from build123d import *

# Parameters (mm, degrees)
SKETCH1_W           = 600
SKETCH1_H           = 300
BOSS_EXTRUDE1_DEPTH = 60
SKETCH2_R           = 42.5
SKETCH2_W           = 550
SKETCH2_H           = 60
CUT_EXTRUDE1_DEPTH  = 34
SKETCH3_W           = 580
SKETCH3_H           = 280
CUT_EXTRUDE2_DEPTH  = 4
SKETCH4_W           = 15
SKETCH4_H           = 96.703930486
CUT_EXTRUDE3_DEPTH  = 4
LPATTERN1_COUNT     = 3
LPATTERN1_PITCH     = 100
LPATTERN1_COL_COUNT = 3
LPATTERN1_COL_PITCH = 100


with BuildPart() as part:
    # Sketch1 → Boss-Extrude1 (new body)
    with BuildSketch(Plane(origin=(0, 0, 0), x_dir=(1, 0, 0), z_dir=(0, 1, 0))):
        Rectangle(SKETCH1_W, SKETCH1_H)
    extrude(amount=BOSS_EXTRUDE1_DEPTH)

    # Sketch2 → Cut-Extrude1 (cut)
    with BuildSketch(Plane(origin=(0, 60, 0), x_dir=(1, 0, 0), z_dir=(0, 1, 0))):
        with Locations(Location((0, 80, 0), (0, 0, 270))):
            Circle(SKETCH2_R)
        with Locations(Location((0, -80, 0), (0, 0, 90))):
            Circle(SKETCH2_R)
        with Locations(Location((-100, 80, 0), (0, 0, 270))):
            Circle(SKETCH2_R)
        with Locations(Location((-200, 80, 0), (0, 0, 270))):
            Circle(SKETCH2_R)
        with Locations(Location((200, 80, 0), (0, 0, 90))):
            Circle(SKETCH2_R)
        with Locations(Location((100, 80, 0), (0, 0, 90))):
            Circle(SKETCH2_R)
        with Locations(Location((200, -80, 0), (0, 0, 270))):
            Circle(SKETCH2_R)
        with Locations(Location((100, -80, 0), (0, 0, 270))):
            Circle(SKETCH2_R)
        with Locations(Location((-100, -80, 0), (0, 0, 90))):
            Circle(SKETCH2_R)
        with Locations(Location((-200, -80, 0), (0, 0, 90))):
            Circle(SKETCH2_R)
        Rectangle(SKETCH2_W, SKETCH2_H)
    extrude(amount=-CUT_EXTRUDE1_DEPTH, mode=Mode.SUBTRACT)

    # Sketch3 → Cut-Extrude2 (cut)
    with BuildSketch(Plane(origin=(0, 60, 0), x_dir=(1, 0, 0), z_dir=(0, 1, 0))):
        Rectangle(SKETCH3_W, SKETCH3_H)
    extrude(amount=-CUT_EXTRUDE2_DEPTH, mode=Mode.SUBTRACT)

    # Sketch4 → Cut-Extrude3 (cut)
    with BuildSketch(Plane(origin=(0, 56, 0), x_dir=(1, 0, 0), z_dir=(0, 1, 0))):
        Rectangle(SKETCH4_W, SKETCH4_H)
    cut_extrude3 = extrude(amount=-CUT_EXTRUDE3_DEPTH, mode=Mode.SUBTRACT)

    # LPattern1: Cut-Extrude3 ×3
    with Locations(*[(-i * LPATTERN1_PITCH, 0, 0) for i in range(1, LPATTERN1_COUNT)]):
        add(cut_extrude3, mode=Mode.SUBTRACT)

    # LPattern1 col: Cut-Extrude3 ×3
    with Locations(*[(i * LPATTERN1_COL_PITCH, 0, 0) for i in range(1, LPATTERN1_COL_COUNT)]):
        add(cut_extrude3, mode=Mode.SUBTRACT)


solid = part.part
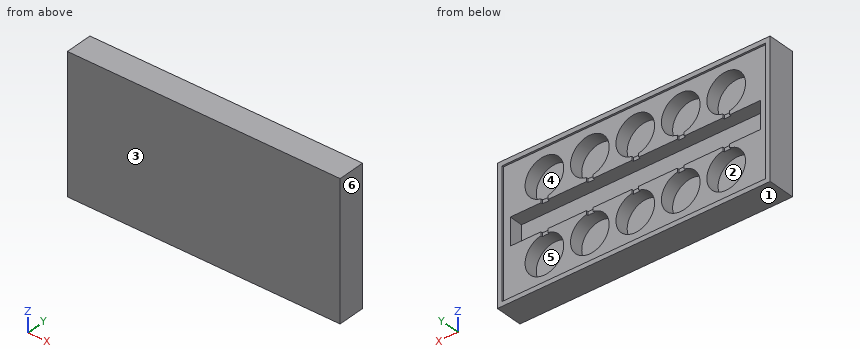
Verification items for the finished model (mm, model axes). Face numbers are marked on the shaded views. A direction names the side the tool comes from. Round coordinates to 2 decimals unless told otherwise and drop trailing zeros. Loops run counter-clockwise (first coordinate to the right, second up) from the corner with the lowest first, then second, coordinate; pieces in that order, holes last. Notation, with made-up numbers: (68.25, 0) - (117.25, 0) arc R22 ccw to (117.25, 11) - close; hole circle Ø10 at (65, 36). An arc over 180 degrees is marked (long way). Answer in a Markdown table with one row per item. Add a question column.
Q1. Release check for a two-part mould opening along Z. For the marked faces 1, 2, 3 and 4 record: pulls with the +Z half, pulls with the -Z half, needs draft (parallel to the pull), parting line crosses it, or undercut.
Q2. Section check D-D on z = 23.5. Enter the section's corners in (x, y), plus the area to 3 significant figures.
Q3. Section check C-C on x = -100. Enter the section's corners in (y, z).
Q4. Tool access check on the marked faces 5 and 6. Record the directions out of +Z, -Z, +X, -X, +Y, -Y that give a thin tool (end or side, any length) a straight path to the whole face; none if there is none.
Q5. Section check A-A on y = 33. State how many separate pieces and enclosed holes the cut face has, plus the area to 3 significant figures.
Q6. Material ranges on line 1 (X direction, y = 37, z = -80); line 2 (X direction, y = 42, z = -77); line 3 (Z direction, x = -68.5, y = 41.5), recorded low to high.
Q7. Gauge pin test, flat ends, axial feed: pin 1 (9 mm diameter, centred on x = -98.5, z = 33.5, fed in from +Y); pin 2 (12 mm diameter, centred on x = -104.5, z = 77, fed in from +Y); pin 3 (6 mm diameter, centred on x = -230, z = -17.5, fed in from -Y). Record the tip position at first contact, or that the pin passes through.
Q8. Section check B-B on z = -80. Enter the section's corners in (x, y).
Found:
| question | item | result |
|---|---|---|
| 1 | face 1 | pulls with the -Z half |
| 1 | face 2 | undercut |
| 1 | face 3 | needs draft |
| 1 | face 4 | undercut |
| 2 | outline | (-300, 0) - (300, 0) - (300, 60) - (290, 60) - (290, 56) - (275, 56) - (275, 26) - (-275, 26) - (-275, 56) - (-290, 56) - (-290, 60) - (-300, 60) - close |
| 2 | area | 17,200 mm² |
| 3 | outline | (0, -150) - (60, -150) - (60, -140) - (56, -140) - (56, -122.5) - (26, -122.5) - (26, -37.5) - (52, -37.5) - (52, -30) - (26, -30) - (26, 30) - (52, 30) - (52, 37.5) - (26, 37.5) - (26, 122.5) - (56, 122.5) - (56, 140) - (60, 140) - (60, 150) - (0, 150) - close |
| 4 | face 5 | +Y |
| 4 | face 6 | +Z, -Z, +X, +Y, -Y |
| 5 | separate pieces | 1 |
| 5 | enclosed holes | 11 |
| 5 | area | 90,300 mm² |
| 6 | line 1 | x = -300 to -242.5, -157.5 to -142.5, -57.5 to -42.5, 42.5 to 57.5, 142.5 to 157.5, 242.5 to 300 |
| 6 | line 2 | x = -300 to -242.39, -157.61 to -142.39, -57.61 to -42.39, 42.39 to 57.61, 142.39 to 157.61, 242.39 to 300 |
| 6 | line 3 | z = -150 to -108.53, -51.47 to -30, 30 to 51.47, 108.53 to 150 |
| 7 | pin 1 | stops at y = 52 |
| 7 | pin 2 | stops at y = 26 |
| 7 | pin 3 | stops at y = 0 |
| 8 | outline | (-300, 0) - (300, 0) - (300, 60) - (290, 60) - (290, 56) - (242.5, 56) - (242.5, 26) - (157.5, 26) - (157.5, 56) - (142.5, 56) - (142.5, 26) - (57.5, 26) - (57.5, 56) - (42.5, 56) - (42.5, 26) - (-42.5, 26) - (-42.5, 56) - (-57.5, 56) - (-57.5, 26) - (-142.5, 26) - (-142.5, 56) - (-157.5, 56) - (-157.5, 26) - (-242.5, 26) - (-242.5, 56) - (-290, 56) - (-290, 60) - (-300, 60) - close |
